from build123d import *

# Parameters (mm, degrees)
SKETCH1_R           = 40
SKETCH1_R_2         = 30
BOSS_EXTRUDE1_DEPTH = 11.5
CHAMFER1_SIZE       = 1


with BuildPart() as part:
    # Sketch1 → Boss-Extrude1 (new, symmetric)
    with BuildSketch(Plane.XY):
        Circle(SKETCH1_R)
        Circle(SKETCH1_R_2, mode=Mode.SUBTRACT)
    extrude(amount=BOSS_EXTRUDE1_DEPTH, both=True)

    # Chamfer1
    chamfer1_edges = [part.edges().sort_by_distance(p)[0] for p in [
        (-40, 0, -11.5),
        (-40, 0, 11.5),
        (-30, 0, -11.5),
        (-30, 0, 11.5),
    ]]
    chamfer(chamfer1_edges, length=CHAMFER1_SIZE)


solid = part.part
For this review, take the finished solid that the model builds, in its own axes (mm). Coordinates: 2 decimals unless noted, no trailing zeros. Loops run counter-clockwise (first coordinate to the right, second up) from the corner with the lowest first, then second, coordinate; pieces in that order, holes last. Notation, with made-up numbers: (88.25, 63.5) - (131.25, 63.5) arc R23 ccw to (131.25, 74.5) - close; hole circle Ø3 at (-6, 69). An arc over 180 degrees is marked (long way). Use a Markdown table: item, result. Add a question column.
Item 1: We need section A-A (x = 0). Give the boundary of the cut face in (y, z).
Item 2: Mouldability with a two-part tool opening along Y and no side actions: class faces 1 (the face through (-29.97, 1.32, -0.15)), 2 (the face through (-26.2, -17.2, 11.5)), 3 (the face through (-8.67, -39.05, 0.15)) as pulls with the +Y half, pulls with the -Y half, needs draft (parallel to the pull), parting line crosses it, or undercut.
Item 3: Insertion check: pin 1 Ø4 at (y, z) = (28.5, -8) entering from -X; pin 2 Ø12 at (y, z) = (25.5, 0.5) entering from +X; pin 3 Ø1 at (y, z) = (12.5, 4) entering from +X. Each pin has a flat end and moves straight along its axis. Give the tip position at first contact, or say it passes through.
Item 4: For line 1 (Y direction, x = 0.5, z = 2.5); line 2 (Y direction, x = -5, z = -7.25); line 3 (X direction, y = -19, z = -7.75), list the stretches that pass through material, from the lowest coordinate up.
Item 5: We need section C-C (z = 9). Give the boundary of the cut face in (x, y).
Results list:
| question | item | result |
|---|---|---|
| 1 | outline | (-40, -10.5) - (-39, -11.5) - (-31, -11.5) - (-30, -10.5) - (-30, 10.5) - (-31, 11.5) - (-39, 11.5) - (-40, 10.5) - close; (30, -10.5) - (31, -11.5) - (39, -11.5) - (40, -10.5) - (40, 10.5) - (39, 11.5) - (31, 11.5) - (30, 10.5) - close |
| 2 | face 1 | undercut |
| 2 | face 2 | needs draft |
| 2 | face 3 | parting line crosses it |
| 3 | pin 1 | stops at x = -29.96 |
| 3 | pin 2 | stops at x = 34.92 |
| 3 | pin 3 | stops at x = 38.16 |
| 4 | line 1 | y = -40 to -30, 30 to 40 |
| 4 | line 2 | y = -39.69 to -29.58, 29.58 to 39.69 |
| 4 | line 3 | x = -35.2 to -23.22, 23.22 to 35.2 |
| 5 | outline | circle Ø80 at (0, 0); hole circle Ø60 at (0, 0) |
